Check sheet for the modelled part. Datum: model origin and axes. Units: mm. Face numbers are marked on the shaded views. A direction names the side the tool comes from. Give positions to 0.01 mm unless a question says otherwise; leave off trailing zeros. Write each loop counter-clockwise with the first axis right and the second up, starting at its lowest first coordinate (ties: lowest second). Pieces come first, ordered by that corner, then holes. Notation, with made-up numbers: (-5.5, -35) -> (24.5, -35) arc R15 cw to (24.5, -28) -> close; hole circle Ø7 at (36, 45). An arc over 180 degrees is marked (long way). Use a Markdown table: item, result. Add a question column.
1. Scan lines: probe 1 along Z at (x, y) = (0, 2.5); probe 2 along Y at (x, z) = (2.75, 15); probe 3 along Z at (x, y) = (-1, 1.5). Record each from-to range of solid material in increasing order. Write a range as [from, to].
2. Cross-section at A-A (y = 0). Enter the section's corners in (x, z).
3. Set-up check for the marked faces 1 and 2: record each of +Z, -Z, +X, -X, +Y, -Y from which the full face is reachable in a straight line by a thin tool's end or side.
4. Cross-section at B-B (x = 0). Enter the section's corners in (y, z).
5. Cross-section at C-C (z = 15). Enter the section's corners in (x, y).
6. Gauge pin test, flat ends, axial feed: P1, Ø1.5, axis at x = 0.5, y = -4, coming from the -Z side; P2, Ø5, axis at x = 0, z = 0, coming from the -Y side; P3, Ø1.5, axis at x = -2.5, z = -37.5, coming from the -Y side; P4, Ø1, axis at y = 4, z = -17.5, coming from the +X side. Record the tip position at first contact, or that the pin passes through.
7. Cross-section at D-D (z = -30). Enter the section's corners in (x, y).
from build123d import *

# Parameters (mm, degrees)
SKETCH_1_W          = 13
SKETCH_1_H          = 13
EXTRUDE_1_DEPTH     = 10
SKETCH_3_R          = 3
CUT_EXTRUDE_1_DEPTH = 20
SKETCH_4_R          = 4
EXTRUDE_2_DEPTH     = 75
SKETCH_5_W          = 13
SKETCH_5_H          = 13
EXTRUDE_3_DEPTH     = 15
SKETCH_6_R          = 4
CUT_EXTRUDE_2_DEPTH = 37
SKETCH_7_R          = 2
CUT_EXTRUDE_3_DEPTH = 300


with BuildPart() as part:
    # 草图1 → 凸台-拉伸1 (new, symmetric)
    with BuildSketch(Plane.XY):
        Rectangle(SKETCH_1_W, SKETCH_1_H)
    extrude(amount=EXTRUDE_1_DEPTH, both=True)

    # 草图3 → 切除-拉伸1 (cut)
    with BuildSketch(Plane(origin=(0, 6.5, 0), x_dir=(1, 0, 0), z_dir=(0, 1, 0))):
        with Locations(Location((0, 0, 0), (0, 0, 180))):
            Circle(SKETCH_3_R)
    extrude(amount=-CUT_EXTRUDE_1_DEPTH, mode=Mode.SUBTRACT)

    # 草图4 → 凸台-拉伸2 (add)
    with BuildSketch(Plane(origin=(0, 0, -10), x_dir=(-1, 0, 0), z_dir=(0, 0, -1))):
        Circle(SKETCH_4_R)
    extrude(amount=EXTRUDE_2_DEPTH)

    # 草图5 → 凸台-拉伸3 (add)
    with BuildSketch(Plane.XY.offset(10)):
        Rectangle(SKETCH_5_W, SKETCH_5_H)
    extrude(amount=EXTRUDE_3_DEPTH)

    # 草图6 → 切除-拉伸2 (cut)
    with BuildSketch(Plane.ZY.offset(6.5)):
        with Locations((15, 0)):
            Circle(SKETCH_6_R)
    extrude(amount=-CUT_EXTRUDE_2_DEPTH, mode=Mode.SUBTRACT)

    # 草图7 → 切除-拉伸3 (cut)
    with BuildSketch(Plane.ZY.offset(6.5)):
        with Locations(Location((-80, 0, 0), (0, 0, 179.999999996))):
            Circle(SKETCH_7_R)
    extrude(amount=-CUT_EXTRUDE_3_DEPTH, mode=Mode.SUBTRACT)


solid = part.part
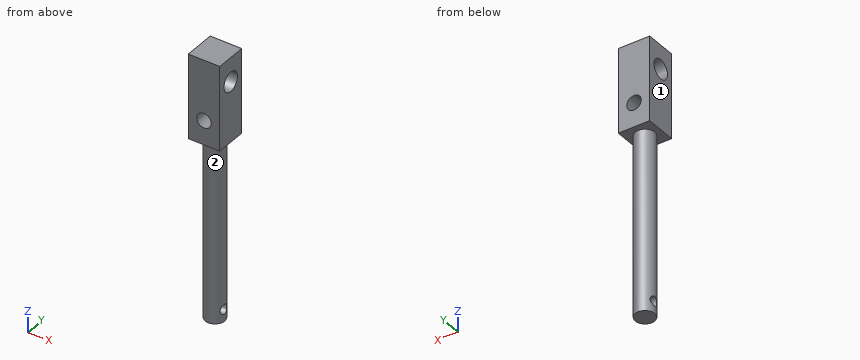
Worked answers:
| question | item | result |
|---|---|---|
| 1 | probe 1 | z = [-85, -3], [3, 11.88], [18.12, 25] |
| 1 | probe 2 | y = [-6.5, -4], [4, 6.5] |
| 1 | probe 3 | z = [-85, -81.32], [-78.68, -2.83], [2.83, 11.29], [18.71, 25] |
| 2 | outline | (-6.5, -10) -> (-4, -10) -> (-4, -78) -> (4, -78) -> (4, -10) -> (6.5, -10) -> (6.5, 11) -> (-6.5, 11) -> close; (-6.5, 19) -> (6.5, 19) -> (6.5, 25) -> (-6.5, 25) -> close; (-4, -85) -> (4, -85) -> (4, -82) -> (-4, -82) -> close; hole circle Ø6 at (0, 0) |
| 3 | face 1 | +Z, -Z, -X, +Y, -Y |
| 3 | face 2 | -Z |
| 4 | outline | (-6.5, -10) -> (-4, -10) -> (-4, -85) -> (4, -85) -> (4, -10) -> (6.5, -10) -> (6.5, -3) -> (-6.5, -3) -> close; (-6.5, 3) -> (6.5, 3) -> (6.5, 25) -> (-6.5, 25) -> close; hole circle Ø8 at (0, 15); hole circle Ø4 at (0, -80) |
| 5 | outline | (-6.5, -6.5) -> (6.5, -6.5) -> (6.5, -4) -> (-6.5, -4) -> close; (-6.5, 4) -> (6.5, 4) -> (6.5, 6.5) -> (-6.5, 6.5) -> close |
| 6 | P1 | stops at z = -85 |
| 6 | P2 | passes through |
| 6 | P3 | stops at y = -3.6 |
| 6 | P4 | stops at x = 1.94 |
| 7 | outline | circle Ø8 at (0, 0) |
